Part model, mm, in its own coordinate system. A direction names the side the tool comes from. Coordinates: 2 decimals unless noted, no trailing zeros. Order: outer loops, then holes, each group sorted by start corner. A loop starts at its lowest first (then second) coordinate and runs counter-clockwise, first axis right, second up.
```python
from build123d import *

# Parameters (mm, degrees)
SKETCH1_W           = 300
SKETCH1_H           = 390
BOSS_EXTRUDE1_DEPTH = 200
SHELL1_T            = -1.5
SKETCH2_W           = 300
SKETCH2_H           = 390
BOSS_EXTRUDE2_DEPTH = 1
SKETCH3_W           = 280
SKETCH3_H           = 370
SKETCH3_W_2         = 276
SKETCH3_H_2         = 366
SKETCH3_R           = 11.25
SKETCH3_W_3         = 24
SKETCH3_H_3         = 80
SKETCH3_W_4         = 45
SKETCH3_H_4         = 45
CUT_EXTRUDE1_DEPTH  = 0.5


with BuildPart() as part:
    # Sketch1 → Boss-Extrude1 (new body)
    with BuildSketch(Plane.XY):
        with Locations((150, 195)):
            Rectangle(SKETCH1_W, SKETCH1_H)
    extrude(amount=BOSS_EXTRUDE1_DEPTH)

    # Shell1
    shell1_openings = [part.faces().sort_by_distance(p)[0] for p in [
        (150, 195, 200),
    ]]
    offset(amount=SHELL1_T, openings=shell1_openings, kind=Kind.INTERSECTION)

    # Sketch2 → Boss-Extrude2 (add)
    with BuildSketch(Plane.XY.offset(200)):
        with Locations((150, 195)):
            Rectangle(SKETCH2_W, SKETCH2_H)
    extrude(amount=BOSS_EXTRUDE2_DEPTH)

    # Sketch3 → Cut-Extrude1 (cut)
    # profile 1 of 5: a face of its own
    with BuildSketch(Plane.XY.offset(201)):
        with Locations((150, 195)):
            Rectangle(SKETCH3_W, SKETCH3_H)
        with Locations((150, 195)):
            Rectangle(SKETCH3_W_2, SKETCH3_H_2, mode=Mode.SUBTRACT)
    # profile 2 of 5: a face of its own
    with BuildSketch(Plane.XY.offset(201)):
        with Locations((150, 247)):
            Circle(SKETCH3_R)
    # profile 3 of 5: a face of its own
    with BuildSketch(Plane.XY.offset(201)):
        with Locations((150, 147)):
            Circle(SKETCH3_R)
    # profile 4 of 5: a face of its own
    with BuildSketch(Plane.XY.offset(201)):
        with Locations((39, 195)):
            Rectangle(SKETCH3_W_3, SKETCH3_H_3)
    # profile 5 of 5: a face of its own
    with BuildSketch(Plane.XY.offset(201)):
        with Locations((150, 325.5)):
            Rectangle(SKETCH3_W_4, SKETCH3_H_4)
    extrude(amount=-CUT_EXTRUDE1_DEPTH, mode=Mode.SUBTRACT)


solid = part.part
```
(1) Tool access for faces 1 (the face through (156.048, 156.486, 200.754)), 2 (the face through (148, 198, 1.5)), 3 (the face through (148, 390, 99)): list every direction of +Z, -Z, +X, -X, +Y, -Y with a clear straight run to the whole face (end or side of a thin tool).
(2) Pull direction X, two halves, no side cores. Call faces 4 (the face through (150, 147, 200.5)), 5 (the face through (39, 196, 200.5)), 6 (the face through (300, 192, 99)), 7 (the face through (148, 198, 201)): +X half, -X half, draft (parallel to the pull), parting line (faces both ways), or undercut.
(3) Slice it at D-D, the plane x = 166.5. Give the cut face in (y, z).
(4) Slice it at B-B, the plane y = 292.5. Give the cut face in (x, z), then the cut area to 3 significant figures.
(5) Probe line 1 (Y direction, x = 185, z = 183); line 2 (Z direction, x = 181.5, y = 307); line 3 (X direction, y = 29, z = 62). List the from-to ranges inside material, lowest first.
(6) Slice it at C-C, the plane z = 150. Give the cut face in (x, y), then the cut area to 3 significant figures.
(7) Slice it at A-A, the plane x = 281.5. Give the cut face in (y, z), then the cut area to 3 significant figures.
Here are the results:
1. face 1: +Z
1. face 2: none
1. face 3: +Z, -Z, +X, -X, +Y
2. face 4: undercut
2. face 5: undercut
2. face 6: +X half
2. face 7: draft
3. outline: (0, 0) - (390, 0) - (390, 201) - (380, 201) - (380, 200.5) - (378, 200.5) - (378, 201) - (348, 201) - (348, 200.5) - (303, 200.5) - (303, 201) - (12, 201) - (12, 200.5) - (10, 200.5) - (10, 201) - (0, 201) - close; hole (1.5, 1.5) - (388.5, 1.5) - (388.5, 200) - (1.5, 200) - close
4. outline: (0, 0) - (300, 0) - (300, 201) - (290, 201) - (290, 200.5) - (288, 200.5) - (288, 201) - (12, 201) - (12, 200.5) - (10, 200.5) - (10, 201) - (0, 201) - close; hole (1.5, 1.5) - (298.5, 1.5) - (298.5, 200) - (1.5, 200) - close
4. area: 1,340 mm2
5. line 1: y = 0 to 1.5, 388.5 to 390
5. line 2: z = 0 to 1.5, 200 to 201
5. line 3: x = 0 to 1.5, 298.5 to 300
6. outline: (0, 0) - (300, 0) - (300, 390) - (0, 390) - close; hole (1.5, 1.5) - (298.5, 1.5) - (298.5, 388.5) - (1.5, 388.5) - close
6. area: 2,060 mm2
7. outline: (0, 0) - (390, 0) - (390, 201) - (380, 201) - (380, 200.5) - (378, 200.5) - (378, 201) - (12, 201) - (12, 200.5) - (10, 200.5) - (10, 201) - (0, 201) - close; hole (1.5, 1.5) - (388.5, 1.5) - (388.5, 200) - (1.5, 200) - close
7. area: 1,570 mm2
